```python
from build123d import *

# Parameters (mm, degrees)
SKETCH_1_W                = 30
SKETCH_1_H                = 352
EXTRUDE_1_DEPTH           = 15
HOLE_WIZARD_1_D           = 6.6
HOLE_WIZARD_1_CBORE_D     = 11
HOLE_WIZARD_1_CBORE_DEPTH = 6.8
FILLET_1_R                = 10


with BuildPart() as part:
    # 草图1 → 凸台-拉伸1 (new body)
    with BuildSketch(Plane.XY):
        Rectangle(SKETCH_1_W, SKETCH_1_H)
    extrude(amount=EXTRUDE_1_DEPTH)

    # 打孔尺寸(%根据)内六角圆柱头螺钉的类型1 (through all)
    with Locations(Plane(origin=(0, 0, 0), x_dir=(-1, 0, 0), z_dir=(0, 0, -1))):
        with Locations((0, 126), (0, -4), (0, -134)):
            CounterBoreHole(HOLE_WIZARD_1_D / 2, HOLE_WIZARD_1_CBORE_D / 2, HOLE_WIZARD_1_CBORE_DEPTH)

    # 圆角1
    fillet_1_edges = [part.edges().sort_by_distance(p)[0] for p in [
        (0, 176, 0),
    ]]
    fillet(fillet_1_edges, radius=FILLET_1_R)


solid = part.part
```
Design review of the part built by this model. Coordinates are the model's own, in mm. A direction names the side the tool comes from. Coordinates: 2 decimals unless noted, no trailing zeros. Order: outer loops, then holes, each group sorted by start corner. A loop starts at its lowest first (then second) coordinate and runs counter-clockwise, first axis right, second up. Notation, with made-up numbers: (-8, 19) - (25, 19) arc R33 cw to (25, 56) - close; hole circle Ø3 at (61, 69.5). An arc over 180 degrees is marked (long way). Answer in a Markdown table with one row per item.
(1) Clearance check with a flat-ended pin moving along its axis: pin 1 (5.5 mm diameter, centred on x = -2.5, y = -4, fed in from -Z). State where the tip first meets the part, or that it passes through.
Checked values:
| item | result |
|---|---|
| pin 1 | z = 6.8 |
(2) Wall thickness on line 1 along Y through (x, z) = (0, 11.75); line 2 along Y through (x, z) = (0, 2.25); line 3 along X through (y, z) = (-134, 13): over which ranges is each line inside the solid? List them lowest first. Write a range as from..to.
Checked values:
| item | result |
|---|---|
| line 1 | -176..-137.3, -130.7..-7.3, -0.7..122.7, 129.3..176 |
| line 2 | -176..-139.5, -128.5..-9.5, 1.5..120.5, 131.5..172.32 |
| line 3 | -15..-3.3, 3.3..15 |
(3) Consider section B-B on z = 4. State the section outline as (x, y) points.
Checked values:
| item | result |
|---|---|
| outline | (-15, -176) - (15, -176) - (15, 174) - (-15, 174) - close; hole circle Ø11 at (0, -134); hole circle Ø11 at (0, -4); hole circle Ø11 at (0, 126) |
(4) For faces 1 (the cylindrical face through (0.716, 131.453, 3.352)), 2 (the cylindrical face through (0.21, 173.15, 3.01)), list the 3-axis set-ups (+Z, -Z, +X, -X, +Y, -Y) from which the entire face can be reached by the end or side of a thin tool; tool diameter is ignored.
Checked values:
| item | result |
|---|---|
| face 1 | -Z |
| face 2 | -Z, +X, -X, +Y |
(5) Consider section C-C on x = 0. Give the number of separate pieces and of enclosed holes in the cut face, plus the area to 3 significant figures.
Checked values:
| item | result |
|---|---|
| separate pieces | 4 |
| enclosed holes | 0 |
| area | 4,870 mm^2 |
(6) The part is to be moulded in two halves that separate along Y. For faces 3 (the flat face through (15, -2, 7)), 4 (the flat face through (0, -176, 7)), 5 (the cylindrical face through (-2.43, -1.77, 10.96)), say which applies: released by +Y, released by -Y, zero draft, split by the parting line, or undercut.
Checked values:
| item | result |
|---|---|
| face 3 | zero draft |
| face 4 | released by -Y |
| face 5 | undercut |
(7) Consider section A-A on y = 126. State the section outline as (x, z) points.
Checked values:
| item | result |
|---|---|
| outline | (-15, 0) - (-5.5, 0) - (-5.5, 6.8) - (-3.3, 6.8) - (-3.3, 15) - (-15, 15) - close; (3.3, 6.8) - (5.5, 6.8) - (5.5, 0) - (15, 0) - (15, 15) - (3.3, 15) - close |
